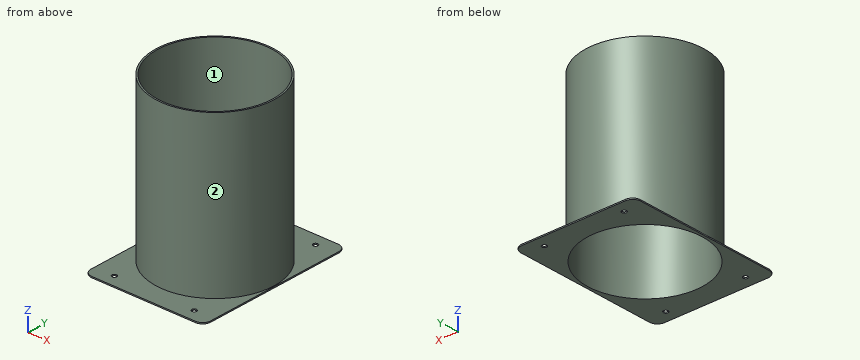
from build123d import *

# Parameters (mm, degrees)
SKETCH_1_R            = 74
SKETCH_1_R_2          = 72
EXTRUDE_1_DEPTH       = 200
SKETCH_2_W            = 150
SKETCH_2_H            = 200
SKETCH_2_R            = 74
EXTRUDE_2_DEPTH       = 1.5
FILLET_1_R            = 10
HOLE_WIZARD_6_0_6_1_D = 6


with BuildPart() as part:
    # 草图1 → 凸台-拉伸1 (new body)
    with BuildSketch(Plane.XY):
        Circle(SKETCH_1_R)
        Circle(SKETCH_1_R_2, mode=Mode.SUBTRACT)
    extrude(amount=EXTRUDE_1_DEPTH)

    # 草图2 → 凸台-拉伸2 (add)
    with BuildSketch(Plane(origin=(0, 0, 0), x_dir=(-1, 0, 0), z_dir=(0, 0, -1))):
        Rectangle(SKETCH_2_W, SKETCH_2_H)
        Circle(SKETCH_2_R, mode=Mode.SUBTRACT)
    extrude(amount=-EXTRUDE_2_DEPTH)

    # 圆角1
    fillet_1_edges = [part.edges().sort_by_distance(p)[0] for p in [
        (-75, 100, 0.75),
        (-75, -100, 0.75),
        (75, -100, 0.75),
        (75, 100, 0.75),
    ]]
    fillet(fillet_1_edges, radius=FILLET_1_R)

    # Ø6.0 (6) 直径孔1 (through all)
    with Locations(Plane.XY.offset(1.5)):
        with Locations((-50, -85), (-50, 85), (50, 85), (50, -85)):
            Hole(HOLE_WIZARD_6_0_6_1_D / 2)


solid = part.part
The listing builds one solid part. Answer for the finished solid, in the listing's coordinates (mm). Face numbers are marked on the shaded views. A direction names the side the tool comes from. Coordinates: 2 decimals unless noted, no trailing zeros. Write each loop counter-clockwise with the first axis right and the second up, starting at its lowest first coordinate (ties: lowest second). Pieces come first, ordered by that corner, then holes. Notation, with made-up numbers: (-29, 57.5) - (-21, 57.5) arc R19 cw to (-21, 90.5) - close; hole circle Ø7 at (-23, 37). An arc over 180 degrees is marked (long way). Return JSON: item names as keys, results as strings.
1. The part is cut by section A-A on y = 0. Determine the outline of the cut face in (x, z), then the cut area to 3 significant figures.
Final values:
{"outline": "(-75, 0) - (-72, 0) - (-72, 200) - (-74, 200) - (-74, 1.5) - (-75, 1.5) - close; (72, 0) - (75, 0) - (75, 1.5) - (74, 1.5) - (74, 200) - (72, 200) - close", "area": "803 mm^2"}
2. The part is cut by section C-C on y = 85. Determine the outline of the cut face in (x, z), then the cut area to 3 significant figures.
Final values:
{"outline": "(-75, 0) - (-53, 0) - (-53, 1.5) - (-75, 1.5) - close; (-47, 0) - (47, 0) - (47, 1.5) - (-47, 1.5) - close; (53, 0) - (75, 0) - (75, 1.5) - (53, 1.5) - close", "area": "207 mm^2"}
3. Consider line 1 along Y through (x, z) = (1, 70); line 2 along Y through (x, z) = (-50, 0.5); line 3 along Z through (x, y) = (-46, -91). Determine where each line is inside the solid, lowest interval first.
Final values:
{"line 1": "-73.99 to -71.99, 71.99 to 73.99", "line 2": "-100 to -88, -82 to -51.81, 51.81 to 82, 88 to 100", "line 3": "0 to 1.5"}
4. Each of these flat-tipped pins is pushed along its axis until it touches: pin 1 Ø4 at (x, z) = (40, 30) entering from -Y; pin 2 Ø5 at (x, y) = (50, 85) entering from -Z; pin 3 Ø4 at (y, z) = (-51.5, 133.5) entering from -X; pin 4 Ø10 at (x, y) = (-27, -78.5) entering from +Z. Where does it stop, or does it pass through?
Final values:
{"pin 1": "y = -63.5", "pin 2": "through", "pin 3": "x = -55.01", "pin 4": "z = 1.5"}
5. Which of the six approach directions +Z, -Z, +X, -X, +Y, -Y give full straight-line access (tool end or side, diameter ignored) to the marked faces 1 and 2?
Final values:
{"face 1": "+Z, -Z", "face 2": "+Z"}
6. The part is cut by section B-B on x = 50. Determine the outline of the cut face in (y, z).
Final values:
{"outline": "(-100, 0) - (-88, 0) - (-88, 1.5) - (-100, 1.5) - close; (-82, 0) - (-51.81, 0) - (-51.81, 200) - (-54.55, 200) - (-54.55, 1.5) - (-82, 1.5) - close; (51.81, 0) - (82, 0) - (82, 1.5) - (54.55, 1.5) - (54.55, 200) - (51.81, 200) - close; (88, 0) - (100, 0) - (100, 1.5) - (88, 1.5) - close"}
7. The part is cut by section D-D on x = 1.5. Determine the outline of the cut face in (y, z).
Final values:
{"outline": "(-100, 0) - (-71.98, 0) - (-71.98, 200) - (-73.98, 200) - (-73.98, 1.5) - (-100, 1.5) - close; (71.98, 0) - (100, 0) - (100, 1.5) - (73.98, 1.5) - (73.98, 200) - (71.98, 200) - close"}
